The listing builds one solid part. Answer for the finished solid, in the listing's coordinates (mm). Face numbers are marked on the shaded views. A direction names the side the tool comes from. Give positions to 0.01 mm unless a question says otherwise; leave off trailing zeros. Loops run counter-clockwise (first coordinate to the right, second up) from the corner with the lowest first, then second, coordinate; pieces in that order, holes last. Notation, with made-up numbers: M -17,-8 L 9,-8 A22 ccw 9,17 Z; hole C 66,-2 d11. An arc over 180 degrees is marked long. One line per item, written item: value. Start each with the question number.
Q1. Flat-ended cylindrical pins translate along their axes: pin 1 (1 mm diameter, centred on x = -54, z = -27.5, fed in from -Y); pin 2 (4 mm diameter, centred on x = -39.5, y = 9.5, fed in from -Z); pin 3 (2 mm diameter, centred on x = 8.5, z = -0.5, fed in from +Y). Find the tip coordinate at first contact, or state that the pin passes through.
Q2. A cutting plane is placed at A-A, the plane y = 2. State how many separate pieces and enclosed holes the cut face has, and give its area (3 significant figures).
Q3. Consider L1, parallel to Z at x = -63, y = 5.75; L2, parallel to Z at x = 7.5, y = 5; L3, parallel to X at y = 4.75, z = -49. Determine where each line is inside the solid, lowest interval first.
Q4. A cutting plane is placed at D-D, the plane z = -41.5. Determine the outline of the cut face in (x, y), and give its area (3 significant figures).
Q5. For the marked faces 1, 2 and 3, determine the directions among +Z, -Z, +X, -X, +Y, -Y from which every point of the face is accessible in a straight line to the end or side of a thin tool.
Q6. The mould has two halves that part along Z. Classify the marked faces 4, 5 and 6: +Z half, -Z half, draft (parallel to the pull), parting line (faces both ways), or undercut.
Q7. A cutting plane is placed at B-B, the plane x = 2. Determine the outline of the cut face in (y, z).
Q8. A cutting plane is placed at C-C, the plane y = 11.5. Determine the outline of the cut face in (x, z), and give its area (3 significant figures).
from build123d import *

# Parameters (mm, degrees)
SKETCH1_W             = 90
SKETCH1_H             = 60
BOSS_EXTRUDE1_DEPTH   = 7.3
SKETCH2_W             = 90
SKETCH2_H             = 11.3
BOSS_EXTRUDE2_DEPTH   = 9.98
M3_TAPPED_HOLE1_D     = 2.5
M3_TAPPED_HOLE1_DEPTH = 7.5
M3_TAPPED_HOLE1_TIP   = 0.751075774
FILLET1_R             = 5
SKETCH5_R             = 3.75
CUT_EXTRUDE1_DEPTH    = 14
SKETCH6_R             = 2.1
CUT_EXTRUDE2_DEPTH    = 94.992651145
SKETCH7_W             = 42
SKETCH7_H             = 0.5
CUT_EXTRUDE3_DEPTH    = 108.961191957
M3_TAPPED_HOLE3_D     = 2.5
M3_TAPPED_HOLE3_DEPTH = 8.5
M3_TAPPED_HOLE3_TIP   = 0.751075774


with BuildPart() as part:
    # Sketch1 → Boss-Extrude1 (new body)
    with BuildSketch(Plane(origin=(0, 0, 0), x_dir=(1, 0, 0), z_dir=(0, 1, 0))):
        with Locations((-28.359375, 27.0703125)):
            Rectangle(SKETCH1_W, SKETCH1_H)
    extrude(amount=BOSS_EXTRUDE1_DEPTH)

    # Sketch2 → Boss-Extrude2 (add)
    with BuildSketch(Plane(origin=(0, 7.3, 0), x_dir=(1, 0, 0), z_dir=(0, 1, 0))):
        with Locations((-28.359375, 2.7203125)):
            Rectangle(SKETCH2_W, SKETCH2_H)
    extrude(amount=BOSS_EXTRUDE2_DEPTH)

    # M3 Tapped Hole1
    with Locations(Plane(origin=(0, 7.3, 0), x_dir=(1, 0, 0), z_dir=(0, 1, 0))):
        with Locations((-66.259375, 19.0703125), (-38.259375, 19.0703125), (-56.759375, 51.5503125), (-43.759375, 51.5503125), (-5.619375, 48.3003125), (7.380625, 48.3003125), (-11.619375, 17.7503125), (9.380625, 17.7503125)):
            Hole(M3_TAPPED_HOLE1_D / 2, depth=M3_TAPPED_HOLE1_DEPTH)
            with Locations((0, 0, -(M3_TAPPED_HOLE1_DEPTH + M3_TAPPED_HOLE1_TIP / 2))):  # 118° drill point
                Cone(0, M3_TAPPED_HOLE1_D / 2, M3_TAPPED_HOLE1_TIP, mode=Mode.SUBTRACT)

    # Fillet1
    fillet1_edges = [part.edges().sort_by_distance(p)[0] for p in [
        (-73.359375, 3.65, -57.0703125),
        (16.640625, 3.65, -57.0703125),
        (16.640625, 8.64, 2.9296875),
        (-73.359375, 8.64, 2.9296875),
    ]]
    fillet(fillet1_edges, radius=FILLET1_R)

    # Sketch5 → Cut-Extrude1 (cut)
    with BuildSketch(Plane(origin=(0, 17.28, 0), x_dir=(1, 0, 0), z_dir=(0, 1, 0))):
        with Locations(Location((-28.359375, 52.0703125, 0), (0, 0, 270))):
            Circle(SKETCH5_R)
        with Locations(Location((-63.359375, 2.0703125, 0), (0, 0, 270))):
            Circle(SKETCH5_R)
        with Locations(Location((6.640625, 2.0703125, 0), (0, 0, 90))):
            Circle(SKETCH5_R)
    extrude(amount=-CUT_EXTRUDE1_DEPTH, mode=Mode.SUBTRACT)

    # Sketch6 → Cut-Extrude2 (cut, through all)
    with BuildSketch(Plane(origin=(0, 3.28, 0), x_dir=(1, 0, 0), z_dir=(0, 1, 0))):
        with Locations(Location((-28.359375, 52.0703125, 0), (0, 0, 270))):
            Circle(SKETCH6_R)
        with Locations(Location((-63.359375, 2.0703125, 0), (0, 0, 270))):
            Circle(SKETCH6_R)
        with Locations(Location((6.640625, 2.0703125, 0), (0, 0, 270))):
            Circle(SKETCH6_R)
    extrude(amount=-CUT_EXTRUDE2_DEPTH, mode=Mode.SUBTRACT)

    # Sketch7 → Cut-Extrude3 (cut, through all)
    with BuildSketch(Plane(origin=(16.640625, 0, 0), x_dir=(0, 0, -1), z_dir=(1, 0, 0))):
        with Locations((27.0703125, 0.25)):
            Rectangle(SKETCH7_W, SKETCH7_H)
    extrude(amount=-CUT_EXTRUDE3_DEPTH, mode=Mode.SUBTRACT)

    # M3 Tapped Hole3
    with Locations(Plane(origin=(0, 7.3, 0), x_dir=(1, 0, 0), z_dir=(0, 1, 0))):
        with Locations((-24.569375, 11.7703125), (-24.569375, 16.9703125), (-25.309375, 23.2703125), (-25.309375, 28.4703125)):
            Hole(M3_TAPPED_HOLE3_D / 2, depth=M3_TAPPED_HOLE3_DEPTH)
            with Locations((0, 0, -(M3_TAPPED_HOLE3_DEPTH + M3_TAPPED_HOLE3_TIP / 2))):  # 118° drill point
                Cone(0, M3_TAPPED_HOLE3_D / 2, M3_TAPPED_HOLE3_TIP, mode=Mode.SUBTRACT)


solid = part.part
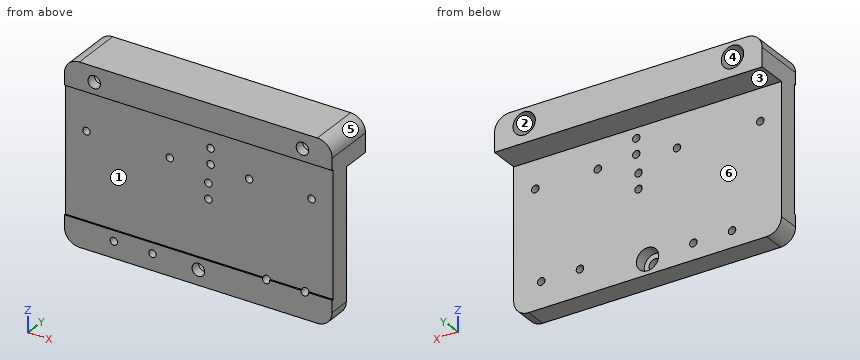
Answer block:
1. pin 1: y = 0.5
1. pin 2: z = -8.37
1. pin 3: y = 3.28
2. separate pieces: 1
2. enclosed holes: 15
2. area: 5,280 mm^2
3. L1: -57.07 to -5.8, 1.66 to 2.93
3. L2: -57.07 to -49.54, -47.06 to -5.72, 1.58 to 2.93
3. L3: -73.36 to -30.51, -26.21 to -6.66, -4.58 to 6.34, 8.42 to 16.64
4. outline: M -73.36,0.5 L 16.64,0.5 L 16.64,7.3 L -73.36,7.3 Z
4. area: 612 mm^2
5. face 1: +X, -X, -Y
5. face 2: +Y
5. face 3: -Z, +X, -X, +Y
6. face 4: undercut
6. face 5: +Z half
6. face 6: draft
7. outline: M 0,-57.07 L 7.3,-57.07 L 7.3,-8.37 L 17.28,-8.37 L 17.28,2.93 L 0,2.93 L 0,-6.07 L 0.5,-6.07 L 0.5,-48.07 L 0,-48.07 Z
8. outline: M -73.36,-8.37 L 16.64,-8.37 L 16.64,-2.07 A5 ccw 11.64,2.93 L -68.36,2.93 A5 ccw -73.36,-2.07 Z; hole C -63.36,-2.07 d7.5; hole C 6.64,-2.07 d7.5
8. area: 918 mm^2
